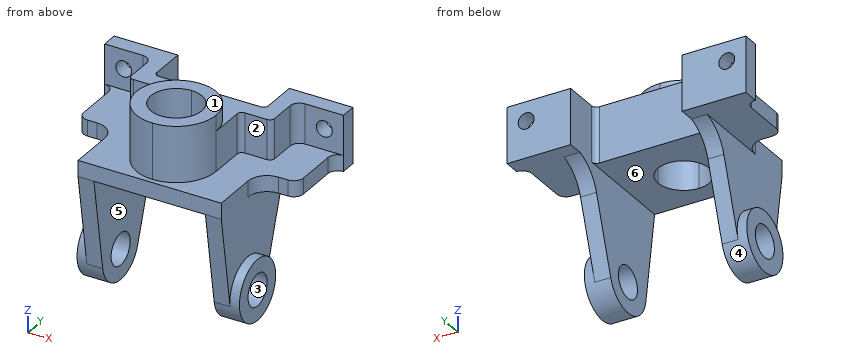
```python
from build123d import *

# Parameters (mm, degrees)
BRACKET_BODY_35MM_DEPTH           = 35
PROFILE_REGION_EXTRUDE_45MM_DEPTH = 45
SLOT_CUT_SKETCH_R                 = 5
SLOT_CUT_DEPTH                    = 45
MOUNTING_PAD_10MM_DEPTH           = 10
EDGE_FILLET_R3_R                  = 3
SIDE_LUG_ARM_10MM_DEPTH           = 10
SKETCH6_3_R                       = 19
SKETCH6_3_R_2                     = 10
SIDE_LUG_BOSS_16MM_DEPTH          = 16


with BuildPart() as part:
    # Bracket Profile Sketch → Bracket Body 35mm (new body)
    with BuildSketch(Plane.XY):
        with BuildLine():
            Line((0, 35), (0, 25))
            ThreePointArc((0, 25), (17.67766953, 17.67766953), (25, 0))
            Line((25, 0), (25, 22))
            ThreePointArc((25, 22), (25.878679656, 24.121320344), (28, 25))
            Line((28, 25), (42, 25))
            ThreePointArc((42, 25), (44.121320344, 25.878679656), (45, 28))
            Line((45, 28), (45, 44))
            ThreePointArc((45, 44), (46.757359313, 48.242640687), (51, 50))
            Line((51, 50), (75, 50))
            Line((75, 50), (75, 60))
            Line((75, 60), (35, 60))
            Line((35, 60), (35, 35))
            Line((35, 35), (0, 35))
        make_face()
        with BuildLine():
            Line((-25, 22), (-25, 0))
            ThreePointArc((-25, 0), (-17.67766953, 17.67766953), (0, 25))
            Line((0, 25), (0, 35))
            Line((0, 35), (-35, 35))
            Line((-35, 35), (-35, 60))
            Line((-35, 60), (-75, 60))
            Line((-75, 60), (-75, 50))
            Line((-75, 50), (-51, 50))
            ThreePointArc((-51, 50), (-46.757359313, 48.242640687), (-45, 44))
            Line((-45, 44), (-45, 28))
            ThreePointArc((-45, 28), (-44.121320344, 25.878679656), (-42, 25))
            Line((-42, 25), (-28, 25))
            ThreePointArc((-28, 25), (-25.878679656, 24.121320344), (-25, 22))
        make_face()
    extrude(amount=BRACKET_BODY_35MM_DEPTH)

    # Sketch1_3 → Profile Region Extrude 45mm (add)
    with BuildSketch(Plane.XY):
        with BuildLine():
            ThreePointArc((0, 25), (-17.67766953, 17.67766953), (-25, 0))
            ThreePointArc((-25, 0), (-17.67766953, -17.67766953), (0, -25))
            Line((0, -25), (0, -16))
            ThreePointArc((0, -16), (-16, 0), (0, 16))
            Line((0, 16), (0, 25))
        make_face()
        with BuildLine():
            ThreePointArc((25, 0), (17.67766953, 17.67766953), (0, 25))
            Line((0, 25), (0, 16))
            ThreePointArc((0, 16), (11.313708499, 11.313708499), (16, 0))
            ThreePointArc((16, 0), (11.313708499, -11.313708499), (0, -16))
            Line((0, -16), (0, -25))
            ThreePointArc((0, -25), (17.67766953, -17.67766953), (25, 0))
        make_face()
        with BuildLine():
            ThreePointArc((0, 25), (-17.67766953, 17.67766953), (-25, 0))
            ThreePointArc((-25, 0), (-17.67766953, -17.67766953), (0, -25))
            Line((0, -25), (0, -16))
            ThreePointArc((0, -16), (-16, 0), (0, 16))
            Line((0, 16), (0, 25))
        make_face()
        with BuildLine():
            ThreePointArc((25, 0), (17.67766953, 17.67766953), (0, 25))
            Line((0, 25), (0, 16))
            ThreePointArc((0, 16), (11.313708499, 11.313708499), (16, 0))
            ThreePointArc((16, 0), (11.313708499, -11.313708499), (0, -16))
            Line((0, -16), (0, -25))
            ThreePointArc((0, -25), (17.67766953, -17.67766953), (25, 0))
        make_face()
    extrude(amount=PROFILE_REGION_EXTRUDE_45MM_DEPTH)

    # Slot Cut Sketch → Slot Cut (cut)
    with BuildSketch(Plane.XZ.offset(-50)):
        with Locations(Location((63, 23, 0), (0, 0, 270))):
            Circle(SLOT_CUT_SKETCH_R)
        with Locations(Location((-63, 23, 0), (0, 0, 270))):
            Circle(SLOT_CUT_SKETCH_R)
    extrude(amount=-SLOT_CUT_DEPTH, mode=Mode.SUBTRACT)

    # Mounting Pad Sketch → Mounting Pad 10mm (add)
    with BuildSketch(Plane(origin=(0, 0, 0), x_dir=(-1, 0, 0), z_dir=(0, 0, -1))):
        with BuildLine():
            Line((51, 50), (75, 50))
            ThreePointArc((75, 50), (70.757359313, 48.242640687), (69, 44))
            Line((69, 44), (69, 18))
            ThreePointArc((69, 18), (67.242640687, 13.757359313), (63, 12))
            Line((63, 12), (57, 12))
            ThreePointArc((57, 12), (48.514718626, 8.485281374), (45, 0))
            Line((45, 0), (45, -28))
            Line((45, -28), (-45, -28))
            Line((-45, -28), (-45, 0))
            ThreePointArc((-45, 0), (-48.514718626, 8.485281374), (-57, 12))
            Line((-57, 12), (-63, 12))
            ThreePointArc((-63, 12), (-67.242640687, 13.757359313), (-69, 18))
            Line((-69, 18), (-69, 44))
            ThreePointArc((-69, 44), (-70.757359313, 48.242640687), (-75, 50))
            Line((-75, 50), (-51, 50))
            ThreePointArc((-51, 50), (-46.757359313, 48.242640687), (-45, 44))
            Line((-45, 44), (-45, 28))
            ThreePointArc((-45, 28), (-44.121320344, 25.878679656), (-42, 25))
            Line((-42, 25), (-28, 25))
            ThreePointArc((-28, 25), (-25.878679656, 24.121320344), (-25, 22))
            Line((-25, 22), (-25, 0))
            ThreePointArc((-25, 0), (0, -25), (25, 0))
            Line((25, 0), (25, 22))
            ThreePointArc((25, 22), (25.878679656, 24.121320344), (28, 25))
            Line((28, 25), (42, 25))
            ThreePointArc((42, 25), (44.121320344, 25.878679656), (45, 28))
            Line((45, 28), (45, 44))
            ThreePointArc((45, 44), (46.757359313, 48.242640687), (51, 50))
        make_face()
    extrude(amount=-MOUNTING_PAD_10MM_DEPTH)

    # Edge Fillet R3
    edge_fillet_r3_edges = [part.edges().sort_by_distance(p)[0] for p in [
        (35, 35, 17.5),
        (-35, 35, 17.5),
    ]]
    fillet(edge_fillet_r3_edges, radius=EDGE_FILLET_R3_R)

    # Side Lug Sketch → Side Lug Arm 10mm (add)
    with BuildSketch(Plane(origin=(-35, 0, 0), x_dir=(0, 0, -1), z_dir=(1, 0, 0))):
        with BuildLine():
            ThreePointArc((58.939212458, -18.771282059), (37.062002462, 1.533704422), (61.921503767, 18.053691953))
            Line((61.921503767, 18.053691953), (16.35266654, 33))
            ThreePointArc((16.35266654, 33), (5.991213295, 39.565558274), (0, 50.269372176))
            Line((0, 50.269372176), (0, 38))
            Line((0, 38), (0, -28))
            Line((0, -28), (58.939212458, -18.771282059))
        make_face()
    side_lug_arm_10mm = extrude(amount=-SIDE_LUG_ARM_10MM_DEPTH)

    # Sketch6_3 → Side Lug Boss 16mm (add)
    with BuildSketch(Plane(origin=(-35, 0, 0), x_dir=(0, 0, -1), z_dir=(1, 0, 0))):
        with Locations((56, 0)):
            Circle(SKETCH6_3_R)
        with Locations((56, 0)):
            Circle(SKETCH6_3_R_2, mode=Mode.SUBTRACT)
    side_lug_boss_16mm = extrude(amount=-SIDE_LUG_BOSS_16MM_DEPTH)

    # Side Lug Mirror: Side Lug Arm 10mm, Side Lug Boss 16mm across plane
    add(side_lug_arm_10mm.mirror(Plane(origin=(0, 0, 0), x_dir=(0, 0, 1), z_dir=(1, 0, 0))))
    add(side_lug_boss_16mm.mirror(Plane(origin=(0, 0, 0), x_dir=(0, 0, 1), z_dir=(1, 0, 0))))


solid = part.part
```
Geometry check sheet. Reference: the model listing, model coordinates, mm. Face numbers are marked on the shaded views. A direction names the side the tool comes from. Coordinates: 2 decimals unless noted, no trailing zeros. Order: outer loops, then holes, each group sorted by start corner. A loop starts at its lowest first (then second) coordinate and runs counter-clockwise, first axis right, second up. Notation, with made-up numbers: M -1.75,38 L 46.25,38 A36 cw 46.25,75 Z; hole C 17.5,23 d11. An arc over 180 degrees is marked long. One line per question, with ' | ' between items. Start each with the question number.
Item 1: Gauge pin test, flat ends, axial feed: pin 1 (3 mm diameter, centred on x = 60.5, z = 5, fed in from -Y); pin 2 (17.5 mm diameter, centred on x = 13, z = 23, fed in from +Y); pin 3 (19 mm diameter, centred on y = -8, z = -59, fed in from +X). Record the tip position at first contact, or that the pin passes through.
Item 2: Cross-section at C-C on z = 23. State how many separate pieces and enclosed holes the cut face has, then the cut area to 3 significant figures.
Item 3: Draft check along Z on the marked faces 1, 2 and 3. Enter one of: pulls with the +Z half, pulls with the -Z half, needs draft (parallel to the pull), parting line crosses it, or undercut.
Item 4: Cross-section at B-B on z = -56. Enter the section's corners in (x, y).
Item 5: Material ranges on L1, parallel to X at y = 57, z = 23; L2, parallel to X at y = 26, z = -30.5; L3, parallel to X at y = 28, z = 29, recorded low to high. Write a range as [from, to].
Item 6: Set-up check for the marked faces 4, 5 and 6: record each of +Z, -Z, +X, -X, +Y, -Y from which the full face is reachable in a straight line by a thin tool's end or side.
Item 7: Cross-section at A-A on x = -38. Enter the section's corners in (y, z).
Findings:
1) pin 1: stops at y = 12 | pin 2: stops at y = 35 | pin 3: stops at x = 51
2) separate pieces: 3 | enclosed holes: 1 | area: 3,250 mm²
3) face 1: pulls with the +Z half | face 2: needs draft | face 3: undercut
4) outline: M -51,-19 L -45,-19 L -45,-19.23 L -35,-19.23 L -35,-10 L -51,-10 Z; M -51,10 L -35,10 L -35,20 L -45,20 L -45,19 L -51,19 Z; M 35,-19.23 L 45,-19.23 L 45,-19 L 51,-19 L 51,-10 L 35,-10 Z; M 35,10 L 51,10 L 51,19 L 45,19 L 45,20 L 35,20 Z
5) L1: x = [-75, -68], [-58, -35], [35, 58], [68, 75] | L2: x = [-45, -35], [35, 45] | L3: x = [-45, 45]
6) face 4: -X | face 5: -Z, +Y | face 6: -Z, +Y, -Y
7) outline: M -28,0 L -18.77,-58.94 A19 ccw 18.05,-61.92 L 33,-16.35 A25 cw 50.27,0 L 60,0 L 60,35 L 25,35 L 25,10 L -28,10 Z; hole C 0,-56 d20
